Read the model definition and answer for the solid it produces. Units are mm, in the model's axes. Face numbers are marked on the shaded views. A direction names the side the tool comes from. Coordinates: 2 decimals unless noted, no trailing zeros. Write each loop counter-clockwise with the first axis right and the second up, starting at its lowest first coordinate (ties: lowest second). Pieces come first, ordered by that corner, then holes. Notation, with made-up numbers: (46.5, 4) -> (66.5, 4) arc R20 cw to (66.5, 19) -> close; hole circle Ø8 at (40.5, 75.25). An arc over 180 degrees is marked (long way). Answer in a Markdown table with one row per item. Add a question column.
Item 1: Section A-A on y = 0 is taken. Write down the section's boundary in (x, z).
Item 2: Section D-D on z = -2.5 is taken. Write down the section's boundary in (x, y).
Item 3: Given pin 1 Ø2 at (x, y) = (2.5, -0.5) entering from +Z; pin 2 Ø2.5 at (x, z) = (54.5, 2) entering from -Y; pin 3 Ø2.5 at (x, z) = (62.5, -2) entering from +Y, each flat-ended and moving along its own axis, determine where each tip first touches the part or whether it passes through.
Item 4: Section B-B on x = 17.5 is taken. Write down the section's boundary in (y, z), then the cut area to 4 significant figures.
Item 5: Section C-C on z = 2.25 is taken. Write down the section's boundary in (x, y), then the cut area to 3 significant figures.
Item 6: Straight lines are drawn through the part: line 1 (X direction, y = -2, z = 2.75); line 2 (Z direction, x = 43, y = 2); line 3 (Y direction, x = 5, z = 2.5). For each, find the intervals that lie inside material, in ascending order. Write a range as from..to.
Item 7: Which of the six approach directions +Z, -Z, +X, -X, +Y, -Y give full straight-line access (tool end or side, diameter ignored) to the marked faces 1 and 2?
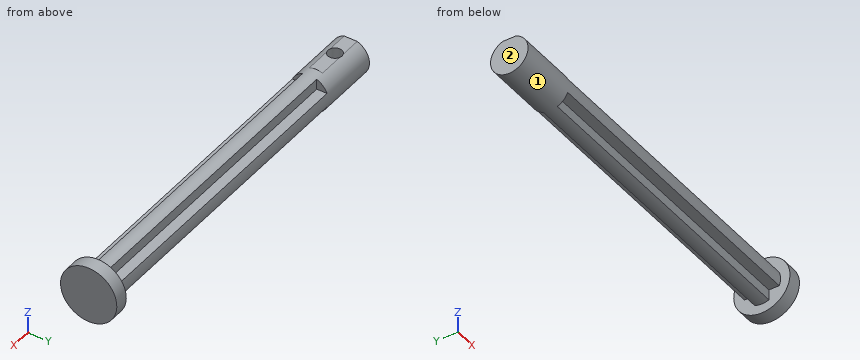
```python
from build123d import *

# Parameters (mm, degrees)
SHANK_PROFILE_8_R           = 4
SHANK_8X80_DEPTH            = 80
SHANK_START                 = -67
SHANK_FLATS_67MM_DEPTH      = 67
HEAD_PROFILE_12_R           = 6
HEAD_12X3_DEPTH             = 3
END_CUT_PROFILE_R           = 1.5
END_POCKET_CUT_4MM_DEPTH    = 4
SKETCH5_4_W                 = 11
SKETCH5_4_H                 = 3
END_RELIEF_CUT_0_25MM_DEPTH = 0.25


with BuildPart() as part:
    # Shank Profile _8 → Shank _8x80 (new body)
    with BuildSketch(Plane(origin=(0, 0, 0), x_dir=(0, 0, -1), z_dir=(1, 0, 0))):
        Circle(SHANK_PROFILE_8_R)
    extrude(amount=SHANK_8X80_DEPTH)

    # Shank Flats Profile → Shank Flats 67mm (cut)
    with BuildSketch(Plane(origin=(80, 0, 0), x_dir=(0, 0, -1), z_dir=(1, 0, 0)).offset(SHANK_START)):
        with BuildLine():
            Line((-1.5, 1.5), (-1.5, 3.708099244))
            ThreePointArc((-1.5, 3.708099244), (-2.828427125, 2.828427125), (-3.708099244, 1.5))
            Line((-3.708099244, 1.5), (-1.5, 1.5))
        make_face()
        with BuildLine():
            Line((1.5, 1.5), (1.5, 3.708099244))
            ThreePointArc((1.5, 3.708099244), (2.828427125, 2.828427125), (3.708099244, 1.5))
            Line((3.708099244, 1.5), (1.5, 1.5))
        make_face()
        with BuildLine():
            Line((1.5, -3.708099244), (1.5, -1.5))
            Line((1.5, -1.5), (3.708099244, -1.5))
            ThreePointArc((3.708099244, -1.5), (2.828427125, -2.828427125), (1.5, -3.708099244))
        make_face()
        with BuildLine():
            Line((-3.708099244, -1.5), (-1.5, -1.5))
            Line((-1.5, -1.5), (-1.5, -3.708099244))
            ThreePointArc((-1.5, -3.708099244), (-2.828427125, -2.828427125), (-3.708099244, -1.5))
        make_face()
    extrude(amount=SHANK_FLATS_67MM_DEPTH, mode=Mode.SUBTRACT)

    # Head Profile _12 → Head _12x3 (add)
    with BuildSketch(Plane(origin=(80, 0, 0), x_dir=(0, 0, -1), z_dir=(1, 0, 0))):
        Circle(HEAD_PROFILE_12_R)
    extrude(amount=HEAD_12X3_DEPTH)

    # End Cut Profile → End Pocket Cut 4mm (cut)
    with BuildSketch(Plane.XY.offset(4)):
        with Locations((5, 0)):
            Circle(END_CUT_PROFILE_R)
    extrude(amount=-END_POCKET_CUT_4MM_DEPTH, mode=Mode.SUBTRACT)

    # Sketch5_4 → End Relief Cut 0.25mm (cut)
    with BuildSketch(Plane.XY.offset(4)):
        with Locations((5.5, 0)):
            Rectangle(SKETCH5_4_W, SKETCH5_4_H)
    extrude(amount=-END_RELIEF_CUT_0_25MM_DEPTH, mode=Mode.SUBTRACT)


solid = part.part
```
Results below:
| question | item | result |
|---|---|---|
| 1 | outline | (0, -4) -> (80, -4) -> (80, -6) -> (83, -6) -> (83, 6) -> (80, 6) -> (80, 4) -> (11, 4) -> (11, 3.75) -> (6.5, 3.75) -> (6.5, 0) -> (3.5, 0) -> (3.5, 3.75) -> (0, 3.75) -> close |
| 2 | outline | (0, -3.12) -> (13, -3.12) -> (13, -1.5) -> (80, -1.5) -> (80, -5.45) -> (83, -5.45) -> (83, 5.45) -> (80, 5.45) -> (80, 1.5) -> (13, 1.5) -> (13, 3.12) -> (0, 3.12) -> close |
| 3 | pin 1 | stops at z = 3.75 |
| 3 | pin 2 | stops at y = -3.93 |
| 3 | pin 3 | stops at y = 3.93 |
| 4 | outline | (-3.71, -1.5) -> (-1.5, -1.5) -> (-1.5, -3.71) arc R4 ccw to (1.5, -3.71) -> (1.5, -1.5) -> (3.71, -1.5) arc R4 ccw to (3.71, 1.5) -> (1.5, 1.5) -> (1.5, 3.71) arc R4 ccw to (-1.5, 3.71) -> (-1.5, 1.5) -> (-3.71, 1.5) arc R4 ccw to start |
| 4 | area | 37.85 mm2 |
| 5 | outline | (0, -3.31) -> (13, -3.31) -> (13, -1.5) -> (80, -1.5) -> (80, -5.56) -> (83, -5.56) -> (83, 5.56) -> (80, 5.56) -> (80, 1.5) -> (13, 1.5) -> (13, 3.31) -> (0, 3.31) -> close; hole circle Ø3 at (5, 0) |
| 5 | area | 313 mm2 |
| 6 | line 1 | x = 0..13, 80..83 |
| 6 | line 2 | z = -1.5..1.5 |
| 6 | line 3 | y = -3.12..-1.5, 1.5..3.12 |
| 7 | face 1 | -X |
| 7 | face 2 | +Z, -Z, -X, +Y, -Y |
